from build123d import *

# Parameters (mm, degrees)
CUT_EXTRUDE_1_REACH      = 136.681
SKETCH_9_W               = 18
SKETCH_9_H               = 10
EXTRUDE_1_DEPTH          = 83
CUT_EXTRUDE_4_REACH      = 165.25
SKETCH_10_R              = 5
CUT_EXTRUDE_5_REACH      = 206.757
CUT_EXTRUDE_5_END_RADIUS = 40
SKETCH_11_R              = 5
SKETCH_12_R              = 8
CUT_EXTRUDE_6_DEPTH      = 10


with BuildPart() as part:
    # 草图1 → 旋转1 (revolve)
    with BuildSketch(Plane.XY, mode=Mode.PRIVATE) as revolve_1_sk:
        Polygon((30.777777778, 50), (30.777777778, 75), (113.777777778, 75), (113.777777778, 0), (93.777777778, 0), (93.777777778, 30), (95.777777778, 32), (95.777777778, 40), (43.777777778, 40), (43.777777778, 50), align=None)
    revolve(revolve_1_sk.sketch.rotate(Axis((-130.37037037, 0, 0), (1, 0, 0)), 90), axis=Axis((-130.37037037, 0, 0), (1, 0, 0)))

    # 草图6 → 切除-拉伸1 (cut, up to next)
    with BuildSketch(Plane(origin=(113.777777778, 0, 0), x_dir=(0, 0, -1), z_dir=(1, 0, 0)), mode=Mode.PRIVATE) as cut_extrude_1_sk1:
        with BuildLine():
            Line((62.5, 41.457809879), (62.5, -41.457809879))
            ThreePointArc((62.5, -41.457809879), (75, 0), (62.5, 41.457809879))
        make_face()
    cut_extrude_1_tool1 = extrude(cut_extrude_1_sk1.sketch, amount=-CUT_EXTRUDE_1_REACH, mode=Mode.PRIVATE) & part.part
    # 草图6 → 切除-拉伸1 (cut, up to next)
    with BuildSketch(Plane(origin=(113.777777778, 0, 0), x_dir=(0, 0, -1), z_dir=(1, 0, 0)), mode=Mode.PRIVATE) as cut_extrude_1_sk2:
        with BuildLine():
            Line((-62.5, 41.457809879), (-62.5, -41.457809879))
            ThreePointArc((-62.5, -41.457809879), (-75, 0), (-62.5, 41.457809879))
        make_face()
    cut_extrude_1_tool2 = extrude(cut_extrude_1_sk2.sketch, amount=-CUT_EXTRUDE_1_REACH, mode=Mode.PRIVATE) & part.part
    add(cut_extrude_1_tool1.solids().sort_by_distance((113.777778, 0, -67.537528))[0], mode=Mode.SUBTRACT)
    add(cut_extrude_1_tool2.solids().sort_by_distance((113.777778, 0, 67.537528))[0], mode=Mode.SUBTRACT)

    # 草图9 → 凸台-拉伸1 (add)
    with BuildSketch(Plane(origin=(113.777777778, 0, 0), x_dir=(0, 0, -1), z_dir=(1, 0, 0))):
        with Locations((-71.5, 5)):
            Rectangle(SKETCH_9_W, SKETCH_9_H)
        with Locations((71.5, 5)):
            Rectangle(SKETCH_9_W, SKETCH_9_H)
    extrude(amount=-EXTRUDE_1_DEPTH)

    # 草图10 → 切除-拉伸4 (cut, up to next)
    with BuildSketch(Plane(origin=(0, 10, 0), x_dir=(1, 0, 0), z_dir=(0, 1, 0)), mode=Mode.PRIVATE) as cut_extrude_4_sk1:
        with Locations(Location((42.277777778, 72.5, 0), (0, 0, 270))):
            Circle(SKETCH_10_R)
    cut_extrude_4_tool1 = extrude(cut_extrude_4_sk1.sketch, amount=-CUT_EXTRUDE_4_REACH, mode=Mode.PRIVATE) & part.part
    # 草图10 → 切除-拉伸4 (cut, up to next)
    with BuildSketch(Plane(origin=(0, 10, 0), x_dir=(1, 0, 0), z_dir=(0, 1, 0)), mode=Mode.PRIVATE) as cut_extrude_4_sk2:
        with Locations(Location((62.277777778, 72.5, 0), (0, 0, 270))):
            Circle(SKETCH_10_R)
    cut_extrude_4_tool2 = extrude(cut_extrude_4_sk2.sketch, amount=-CUT_EXTRUDE_4_REACH, mode=Mode.PRIVATE) & part.part
    # 草图10 → 切除-拉伸4 (cut, up to next)
    with BuildSketch(Plane(origin=(0, 10, 0), x_dir=(1, 0, 0), z_dir=(0, 1, 0)), mode=Mode.PRIVATE) as cut_extrude_4_sk3:
        with Locations(Location((82.277777778, 72.5, 0), (0, 0, 270))):
            Circle(SKETCH_10_R)
    cut_extrude_4_tool3 = extrude(cut_extrude_4_sk3.sketch, amount=-CUT_EXTRUDE_4_REACH, mode=Mode.PRIVATE) & part.part
    # 草图10 → 切除-拉伸4 (cut, up to next)
    with BuildSketch(Plane(origin=(0, 10, 0), x_dir=(1, 0, 0), z_dir=(0, 1, 0)), mode=Mode.PRIVATE) as cut_extrude_4_sk4:
        with Locations(Location((102.277777778, 72.5, 0), (0, 0, 270))):
            Circle(SKETCH_10_R)
    cut_extrude_4_tool4 = extrude(cut_extrude_4_sk4.sketch, amount=-CUT_EXTRUDE_4_REACH, mode=Mode.PRIVATE) & part.part
    # 草图10 → 切除-拉伸4 (cut, up to next)
    with BuildSketch(Plane(origin=(0, 10, 0), x_dir=(1, 0, 0), z_dir=(0, 1, 0)), mode=Mode.PRIVATE) as cut_extrude_4_sk5:
        with Locations(Location((102.277777778, -72.5, 0), (0, 0, 90))):
            Circle(SKETCH_10_R)
    cut_extrude_4_tool5 = extrude(cut_extrude_4_sk5.sketch, amount=-CUT_EXTRUDE_4_REACH, mode=Mode.PRIVATE) & part.part
    # 草图10 → 切除-拉伸4 (cut, up to next)
    with BuildSketch(Plane(origin=(0, 10, 0), x_dir=(1, 0, 0), z_dir=(0, 1, 0)), mode=Mode.PRIVATE) as cut_extrude_4_sk6:
        with Locations(Location((82.277777778, -72.5, 0), (0, 0, 90))):
            Circle(SKETCH_10_R)
    cut_extrude_4_tool6 = extrude(cut_extrude_4_sk6.sketch, amount=-CUT_EXTRUDE_4_REACH, mode=Mode.PRIVATE) & part.part
    # 草图10 → 切除-拉伸4 (cut, up to next)
    with BuildSketch(Plane(origin=(0, 10, 0), x_dir=(1, 0, 0), z_dir=(0, 1, 0)), mode=Mode.PRIVATE) as cut_extrude_4_sk7:
        with Locations(Location((62.277777778, -72.5, 0), (0, 0, 90))):
            Circle(SKETCH_10_R)
    cut_extrude_4_tool7 = extrude(cut_extrude_4_sk7.sketch, amount=-CUT_EXTRUDE_4_REACH, mode=Mode.PRIVATE) & part.part
    # 草图10 → 切除-拉伸4 (cut, up to next)
    with BuildSketch(Plane(origin=(0, 10, 0), x_dir=(1, 0, 0), z_dir=(0, 1, 0)), mode=Mode.PRIVATE) as cut_extrude_4_sk8:
        with Locations(Location((42.277777778, -72.5, 0), (0, 0, 90))):
            Circle(SKETCH_10_R)
    cut_extrude_4_tool8 = extrude(cut_extrude_4_sk8.sketch, amount=-CUT_EXTRUDE_4_REACH, mode=Mode.PRIVATE) & part.part
    add(cut_extrude_4_tool1.solids().sort_by_distance((42.277778, 10, -72.5))[0], mode=Mode.SUBTRACT)
    add(cut_extrude_4_tool2.solids().sort_by_distance((62.277778, 10, -72.5))[0], mode=Mode.SUBTRACT)
    add(cut_extrude_4_tool3.solids().sort_by_distance((82.277778, 10, -72.5))[0], mode=Mode.SUBTRACT)
    add(cut_extrude_4_tool4.solids().sort_by_distance((102.277778, 10, -72.5))[0], mode=Mode.SUBTRACT)
    add(cut_extrude_4_tool5.solids().sort_by_distance((102.277778, 10, 72.5))[0], mode=Mode.SUBTRACT)
    add(cut_extrude_4_tool6.solids().sort_by_distance((82.277778, 10, 72.5))[0], mode=Mode.SUBTRACT)
    add(cut_extrude_4_tool7.solids().sort_by_distance((62.277778, 10, 72.5))[0], mode=Mode.SUBTRACT)
    add(cut_extrude_4_tool8.solids().sort_by_distance((42.277778, 10, 72.5))[0], mode=Mode.SUBTRACT)

    # 切除-拉伸5: up to this cylinder (the profile starts outside it)
    cut_extrude_5_end = Plane(origin=(73.777778, 0, 0), z_dir=(-1, 0, 0)) * Cylinder(CUT_EXTRUDE_5_END_RADIUS, 494.514, mode=Mode.PRIVATE)
    # 草图11 → 切除-拉伸5 (cut, up to the surface)
    with BuildSketch(Plane(origin=(0, 75, 0), x_dir=(1, 0, 0), z_dir=(0, 1, 0)), mode=Mode.PRIVATE) as cut_extrude_5_sk1:
        with Locations(Location((73.777777778, 0, 0), (0, 0, 270))):
            Circle(SKETCH_11_R)
    cut_extrude_5_tool1 = extrude(cut_extrude_5_sk1.sketch, amount=-CUT_EXTRUDE_5_REACH, mode=Mode.PRIVATE) - cut_extrude_5_end
    add(cut_extrude_5_tool1.solids().sort_by_distance((73.777778, 75, 0))[0], mode=Mode.SUBTRACT)

    # 草图12 → 切除-拉伸6 (cut)
    with BuildSketch(Plane(origin=(0, 75, 0), x_dir=(1, 0, 0), z_dir=(0, 1, 0))):
        with Locations(Location((73.777777778, 0, 0), (0, 0, 270))):
            Circle(SKETCH_12_R)
    extrude(amount=-CUT_EXTRUDE_6_DEPTH, mode=Mode.SUBTRACT)


solid = part.part
Read the model definition and answer for the solid it produces. Units are mm, in the model's axes. A direction names the side the tool comes from. Give positions to 0.01 mm unless a question says otherwise; leave off trailing zeros. Write each loop counter-clockwise with the first axis right and the second up, starting at its lowest first coordinate (ties: lowest second). Pieces come first, ordered by that corner, then holes. Notation, with made-up numbers: (25.5, -16.5) - (30.5, -16.5) arc R19 cw to (30.5, 13.5) - close; hole circle Ø5 at (63.5, 53). An arc over 180 degrees is marked (long way). Use CSV: the item, a comma, the result in double quotes. Start each with the question number.
Item 1: The part is cut by section A-A, the plane z = 72.5. Give the vertices of the cut face in (x, y), and give its area (3 significant figures).
Item 2: The part is cut by section D-D, the plane y = 46. Give the vertices of the cut face in (x, z).
Item 3: Consider line 1 (X direction, y = 2, z = 72.5); line 2 (Z direction, x = 104, y = -26); line 3 (X direction, y = 14, z = -17.5). Determine where each line is inside the solid, lowest interval first.
Item 4: The part is cut by section B-B, the plane z = 0. Give the vertices of the cut face in (x, y).
Item 5: For faces 4 (the flat face through (95.778, -27, 18)), 5 (the flat face through (73, 10, -71)), 6 (the cylindrical face through (68.91, 70.07, -6.35)), determine the directions among +Z, -Z, +X, -X, +Y, -Y from which every point of the face is accessible in a straight line to the end or side of a thin tool.
Item 6: The part is cut by section C-C, the plane x = 84.5. Give the vertices of the cut face in (y, z), and give its area (3 significant figures).
Item 7: The mould has two halves that part along Z. Classify faces 1 (the flat face through (73, 0, 72)), 2 (the cylindrical face through (86.494, 5.07, -69.812)), 3 (the flat face through (73, -20, 62.5)): pulls with the +Z half, pulls with the -Z half, needs draft (parallel to the pull), parting line crosses it, or undercut.
Item 8: Flat-ended cylindrical pins translate along their axes: P1, Ø13, axis at x = 82.28, z = 72.5, coming from the -Y side; P2, Ø25, axis at x = 89.5, y = 33, coming from the -Z side; P3, Ø6, axis at x = 102.28, z = -72.5, coming from the -Y side; P4, Ø5, axis at x = 44.5, z = -63, coming from the -Y side. Find the tip coordinate at first contact, or state that the pin passes through.
Taken from the geometry:
1,outline,"(30.78, 0) - (37.28, 0) - (37.28, 10) - (30.78, 10) - close; (47.28, 0) - (57.28, 0) - (57.28, 10) - (47.28, 10) - close; (67.28, 0) - (77.28, 0) - (77.28, 10) - (67.28, 10) - close; (87.28, 0) - (97.28, 0) - (97.28, 10) - (87.28, 10) - close; (107.28, 0) - (113.78, 0) - (113.78, 10) - (107.28, 10) - close"
1,area,"430 mm2"
2,outline,"(30.78, -59.24) - (113.78, -59.24) - (113.78, 59.24) - (30.78, 59.24) - (30.78, 19.6) - (43.78, 19.6) - (43.78, -19.6) - (30.78, -19.6) - close; hole circle Ø10 at (73.78, 0)"
3,line 1,"30.78 to 37.28, 47.28 to 57.28, 67.28 to 77.28, 87.28 to 97.28, 107.28 to 113.78"
3,line 2,"-62.5 to 62.5"
3,line 3,"93.78 to 113.78"
4,outline,"(30.78, -75) - (113.78, -75) - (113.78, 75) - (81.78, 75) - (81.78, 65) - (78.78, 65) - (78.78, 40) - (95.78, 40) - (95.78, 32) - (93.78, 30) - (93.78, -30) - (95.78, -32) - (95.78, -40) - (43.78, -40) - (43.78, -50) - (30.78, -50) - close; (30.78, 50) - (43.78, 50) - (43.78, 40) - (68.78, 40) - (68.78, 65) - (65.78, 65) - (65.78, 75) - (30.78, 75) - close"
5,face 4,"-X"
5,face 5,"-Z, +X, -X, +Y"
5,face 6,"+Y"
6,outline,"(-41.46, -62.5) - (0, -62.5) - (0, -68.02) - (10, -68.02) - (10, -62.5) - (41.46, -62.5) arc R75 ccw to (41.46, 62.5) - (10, 62.5) - (10, 68.02) - (0, 68.02) - (0, 62.5) - (-41.46, 62.5) arc R75 ccw to start; (0, -80.5) - (10, -80.5) - (10, -76.98) - (0, -76.98) - close; (0, 76.98) - (10, 76.98) - (10, 80.5) - (0, 80.5) - close; hole circle Ø80 at (0, 0)"
6,area,"11,400 mm2"
7,face 1,"needs draft"
7,face 2,"undercut"
7,face 3,"pulls with the +Z half"
8,P1,"y = 0"
8,P2,"z = -62.5"
8,P3,"through"
8,P4,"y = -44.33"
